Could you check a few things on this model? Use its own coordinates, in mm. Face numbers are marked on the shaded views. Give positions to 0.01 mm unless a question says otherwise; leave off trailing zeros. Write each loop counter-clockwise with the first axis right and the second up, starting at its lowest first coordinate (ties: lowest second). Pieces come first, ordered by that corner, then holes. Notation, with made-up numbers: (66.5, 37.5) - (90.5, 37.5) arc R9 ccw to (90.5, 51.5) - close; hole circle Ø9 at (86, 55.25). An arc over 180 degrees is marked (long way). Answer in a Markdown table with one row per item.
from build123d import *

# Parameters (mm, degrees)
SKETCH1_R           = 11.5
BOSS_EXTRUDE1_DEPTH = 45.2
SKETCH4_R           = 10.3
CUT_EXTRUDE1_DEPTH  = 44
SKETCH5_R           = 9.8
CUT_EXTRUDE2_DEPTH  = 0.9


with BuildPart() as part:
    # Sketch1 → Boss-Extrude1 (new body)
    with BuildSketch(Plane(origin=(0, 0, 0), x_dir=(1, 0, 0), z_dir=(0, 1, 0))):
        with Locations(Location((0, 0, 0), (0, 0, 270))):
            Circle(SKETCH1_R)
    extrude(amount=BOSS_EXTRUDE1_DEPTH)

    # Sketch4 → Cut-Extrude1 (cut)
    with BuildSketch(Plane(origin=(0, 45.2, 0), x_dir=(1, 0, 0), z_dir=(0, 1, 0))):
        with Locations(Location((0, 0, 0), (0, 0, 270))):
            Circle(SKETCH4_R)
    extrude(amount=-CUT_EXTRUDE1_DEPTH, mode=Mode.SUBTRACT)

    # Sketch5 → Cut-Extrude2 (cut)
    with BuildSketch(Plane.XZ):
        with Locations(Location((0, 0, 0), (0, 0, 270))):
            Circle(SKETCH5_R)
    extrude(amount=-CUT_EXTRUDE2_DEPTH, mode=Mode.SUBTRACT)


solid = part.part
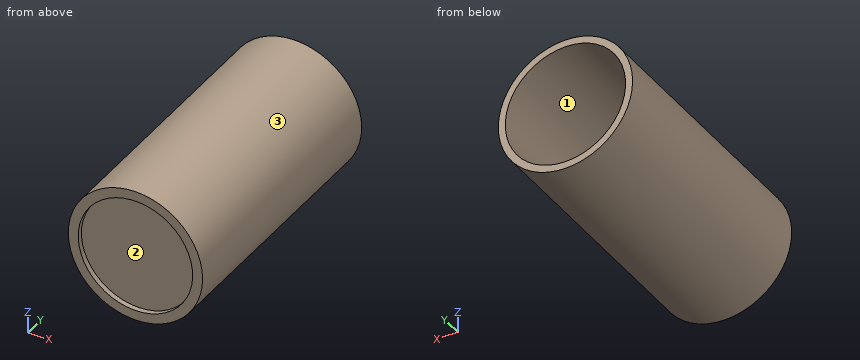
1) We'd pull the mould along X, two halves only. Please class the marked faces 1, 2 and 3: +X half, -X half, draft (parallel to the pull), parting line (faces both ways), or undercut.
Check values:
| item | result |
|---|---|
| face 1 | undercut |
| face 2 | undercut |
| face 3 | parting line |
2) Imagine slicing it at B-B (z = 0). List the corners of the cut face in (x, y) for me.
Check values:
| item | result |
|---|---|
| outline | (-11.5, 0) - (-9.8, 0) - (-9.8, 0.9) - (9.8, 0.9) - (9.8, 0) - (11.5, 0) - (11.5, 45.2) - (10.3, 45.2) - (10.3, 1.2) - (-10.3, 1.2) - (-10.3, 45.2) - (-11.5, 45.2) - close |
3) Imagine slicing it at A-A (x = 0). List the corners of the cut face in (y, z) for me.
Check values:
| item | result |
|---|---|
| outline | (0, -11.5) - (45.2, -11.5) - (45.2, -10.3) - (1.2, -10.3) - (1.2, 10.3) - (45.2, 10.3) - (45.2, 11.5) - (0, 11.5) - (0, 9.8) - (0.9, 9.8) - (0.9, -9.8) - (0, -9.8) - close |
4) Will these pins go through, and if not, where does the flat tip stop? P1, Ø5, axis at y = 7, z = 8, coming from the +X side; P2, Ø1.5, axis at x = -3, z = 8, coming from the -Y side; P3, Ø8, axis at y = 39.5, z = -4.5, coming from the +X side.
Check values:
| item | result |
|---|---|
| P1 | stops at x = 10.1 |
| P2 | stops at y = 0.9 |
| P3 | stops at x = 11.49 |
5) If I drill on line 1 (Z direction, x = -0.25, y = 11); line 2 (X direction, y = 0.6, z = 0), over which ranges is the centre line in solid material (lowest first)?
Check values:
| item | result |
|---|---|
| line 1 | z = -11.5 to -10.3, 10.3 to 11.5 |
| line 2 | x = -11.5 to -9.8, 9.8 to 11.5 |
6) Imagine slicing it at C-C (y = 32.5). List the corners of the cut face in (x, z) for me.
Check values:
| item | result |
|---|---|
| outline | circle Ø23 at (0, 0); hole circle Ø20.6 at (0, 0) |
